```python
from build123d import *

# Parameters (mm, degrees)
SKETCH1_W           = 290
SKETCH1_H           = 350
BOSS_EXTRUDE1_DEPTH = 5
SKETCH2_W           = 114
SKETCH2_H           = 5
BOSS_EXTRUDE2_DEPTH = 81
SKETCH3_W           = 114
SKETCH3_H           = 5
BOSS_EXTRUDE3_DEPTH = 135
FILLET1_R           = 10
SKETCH4_W           = 88
SKETCH4_H           = 15
CUT_EXTRUDE1_DEPTH  = 120
FILLET2_R           = 15
FILLET3_R           = 10
SKETCH5_R           = 4
CUT_EXTRUDE2_DEPTH  = 120
SKETCH7_R           = 2
CUT_EXTRUDE3_DEPTH  = 10
SKETCH8_R           = 3
CUT_EXTRUDE4_DEPTH  = 10
SKETCH9_R           = 4
CUT_EXTRUDE5_DEPTH  = 10
SKETCH10_R          = 2.5
CUT_EXTRUDE6_DEPTH  = 10
SKETCH11_R          = 2.5
CUT_EXTRUDE7_DEPTH  = 10


with BuildPart() as part:
    # Sketch1 → Boss-Extrude1 (new body)
    with BuildSketch(Plane.XY):
        Rectangle(SKETCH1_W, SKETCH1_H)
    extrude(amount=BOSS_EXTRUDE1_DEPTH)

    # Sketch2 → Boss-Extrude2 (add)
    with BuildSketch(Plane.XY.offset(5)):
        with Locations((0, 172.5)):
            Rectangle(SKETCH2_W, SKETCH2_H)
    extrude(amount=-BOSS_EXTRUDE2_DEPTH)

    # Sketch3 → Boss-Extrude3 (add)
    with BuildSketch(Plane(origin=(0, 170, 0), x_dir=(-1, 0, 0), z_dir=(0, -1, 0))):
        with Locations((0, 73.5)):
            Rectangle(SKETCH3_W, SKETCH3_H)
    extrude(amount=-BOSS_EXTRUDE3_DEPTH)

    # Fillet1
    fillet1_edges = [part.edges().sort_by_distance(p)[0] for p in [
        (0, 170, 0),
        (0, 175, -71),
    ]]
    fillet(fillet1_edges, radius=FILLET1_R)

    # Sketch4 → Cut-Extrude1 (cut)
    with BuildSketch(Plane(origin=(0, 0, 0), x_dir=(-1, 0, 0), z_dir=(0, 0, -1))):
        with Locations((101, 167.5)):
            Rectangle(SKETCH4_W, SKETCH4_H)
        with Locations((-101, 167.5)):
            Rectangle(SKETCH4_W, SKETCH4_H)
    extrude(amount=-CUT_EXTRUDE1_DEPTH, mode=Mode.SUBTRACT)

    # Fillet2
    fillet2_edges = [part.edges().sort_by_distance(p)[0] for p in [
        (0, 175, 5),
        (0, 170, -76),
    ]]
    fillet(fillet2_edges, radius=FILLET2_R)

    # Fillet3
    fillet3_edges = [part.edges().sort_by_distance(p)[0] for p in [
        (57, 305, -73.5),
        (-57, 305, -73.5),
    ]]
    fillet(fillet3_edges, radius=FILLET3_R)

    # Sketch5 → Cut-Extrude2 (cut)
    with BuildSketch(Plane(origin=(0, 0, -76), x_dir=(-1, 0, 0), z_dir=(0, 0, -1))):
        with Locations((42, 290)):
            Circle(SKETCH5_R)
        with Locations((-42, 290)):
            Circle(SKETCH5_R)
        with Locations((42, 219)):
            Circle(SKETCH5_R)
        with Locations((-42, 219)):
            Circle(SKETCH5_R)
    extrude(amount=-CUT_EXTRUDE2_DEPTH, mode=Mode.SUBTRACT)

    # Sketch7 → Cut-Extrude3 (cut)
    with BuildSketch(Plane(origin=(0, 0, 0), x_dir=(-1, 0, 0), z_dir=(0, 0, -1))):
        with Locations((-130, -121)):
            Circle(SKETCH7_R)
        with Locations((-65, -121)):
            Circle(SKETCH7_R)
        with Locations((0, -121)):
            Circle(SKETCH7_R)
        with Locations((65, -121)):
            Circle(SKETCH7_R)
        with Locations((130, -121)):
            Circle(SKETCH7_R)
        with Locations((130, -43)):
            Circle(SKETCH7_R)
        with Locations((65, -43)):
            Circle(SKETCH7_R)
        with Locations((0, -43)):
            Circle(SKETCH7_R)
        with Locations((-65, -43)):
            Circle(SKETCH7_R)
        with Locations((-130, -43)):
            Circle(SKETCH7_R)
    extrude(amount=-CUT_EXTRUDE3_DEPTH, mode=Mode.SUBTRACT)

    # Sketch8 → Cut-Extrude4 (cut)
    with BuildSketch(Plane(origin=(0, 0, -76), x_dir=(-1, 0, 0), z_dir=(0, 0, -1))):
        with Locations((-20, 247)):
            Circle(SKETCH8_R)
        with Locations((-20, 263)):
            Circle(SKETCH8_R)
        with Locations((20, 263)):
            Circle(SKETCH8_R)
        with Locations((20, 247)):
            Circle(SKETCH8_R)
    extrude(amount=-CUT_EXTRUDE4_DEPTH, mode=Mode.SUBTRACT)

    # Sketch9 → Cut-Extrude5 (cut)
    with BuildSketch(Plane(origin=(0, 0, 0), x_dir=(-1, 0, 0), z_dir=(0, 0, -1))):
        with Locations((40, -154)):
            Circle(SKETCH9_R)
        with Locations((-40, -154)):
            Circle(SKETCH9_R)
    extrude(amount=-CUT_EXTRUDE5_DEPTH, mode=Mode.SUBTRACT)

    # Sketch10 → Cut-Extrude6 (cut)
    with BuildSketch(Plane(origin=(0, 0, 0), x_dir=(-1, 0, 0), z_dir=(0, 0, -1))):
        with Locations((-135, -165)):
            Circle(SKETCH10_R)
        with Locations((135, -165)):
            Circle(SKETCH10_R)
        with Locations((135, 150)):
            Circle(SKETCH10_R)
        with Locations((-135, 150)):
            Circle(SKETCH10_R)
    extrude(amount=-CUT_EXTRUDE6_DEPTH, mode=Mode.SUBTRACT)

    # Sketch11 → Cut-Extrude7 (cut)
    with BuildSketch(Plane(origin=(0, 0, 0), x_dir=(-1, 0, 0), z_dir=(0, 0, -1))):
        with Locations((135, 110)):
            Circle(SKETCH11_R)
        with Locations((135, 10)):
            Circle(SKETCH11_R)
        with Locations((-135, 110)):
            Circle(SKETCH11_R)
        with Locations((-135, 10)):
            Circle(SKETCH11_R)
    extrude(amount=-CUT_EXTRUDE7_DEPTH, mode=Mode.SUBTRACT)


solid = part.part
```
CAD build for the part. Positions are in the model's coordinates, mm. A direction names the side the tool comes from. Coordinates: 2 decimals unless noted, no trailing zeros. Order: outer loops, then holes, each group sorted by start corner. A loop starts at its lowest first (then second) coordinate and runs counter-clockwise, first axis right, second up.
(1) Saw through at C-C, the plane z = -55. Write the cut outline in (x, y).
Solution:
outline: (-57, 170) - (57, 170) - (57, 175) - (-57, 175) - close
(2) Which spindle directions (+Z, -Z, +X, -X, +Y, -Y) get a long thin tool onto all of the face, cutting with end or side? Do faces 1 (the face through (-1, 175, -36)), 2 (the face through (53.99, 302.15, -73.54)), 3 (the face through (-2, -5, 0)). Say none if no direction does.
Solution:
face 1: +Z, +X, -X, +Y
face 2: +Z, -Z, +X, +Y
face 3: -Z, +X, -X, -Y
(3) Saw through at A-A, the plane x = -30.5. Write the cut outline in (y, z).
Solution:
outline: (-175, 0) - (160, 0) arc R10 cw to (170, -10) - (170, -61) arc R15 ccw to (185, -76) - (305, -76) - (305, -71) - (185, -71) arc R10 cw to (175, -61) - (175, -10) arc R15 ccw to (160, 5) - (-175, 5) - close
(4) Pin check, flat tips, straight feed: pin 1 Ø10 at (x, z) = (23.5, -10) entering from -Y; pin 2 Ø12 at (x, y) = (-104.5, -123) entering from -Z; pin 3 Ø15.5 at (x, z) = (9.5, -34) entering from -Y. Stop position of each tip, or through.
Solution:
pin 1: stops at y = 168.66
pin 2: stops at z = 0
pin 3: stops at y = 170
(5) Drill centre lines: L1, parallel to X at y = 263, z = -74.2; L2, parallel to Y at x = 20, z = -74; L3, parallel to Z at x = 40, y = -15.5. Where is each one in solid material? Low to high.
Solution:
L1: x = -57 to -23, -17 to 17, 23 to 57
L2: y = 177.52 to 244, 250 to 260, 266 to 305
L3: z = 0 to 5
(6) Saw through at B-B, the plane y = 50. Write the cut outline in (x, z), and give its area (3 significant figures).
Solution:
outline: (-145, 0) - (145, 0) - (145, 5) - (-145, 5) - close
area: 1,450 mm2
